Build history of the part. All positions in model axes, mm. A direction names the side the tool comes from. Coordinates: 2 decimals unless noted, no trailing zeros. Write each loop counter-clockwise with the first axis right and the second up, starting at its lowest first coordinate (ties: lowest second). Pieces come first, ordered by that corner, then holes.
```python
from build123d import *

# Parameters (mm, degrees)
BASE_PLATE_SKETCH_145X72_W  = 145
BASE_PLATE_SKETCH_145X72_H  = 72
BASE_PLATE_25_THICK_DEPTH   = 25
UNDERSIDE_RELIEF_SKETCH_W   = 72
UNDERSIDE_RELIEF_SKETCH_H   = 6
UNDERSIDE_RELIEF_CUT_DEPTH  = 50
CLEVIS_SLOT_CUT_DEPTH       = 50
LOCATING_PAD_SKETCH_W       = 12
LOCATING_PAD_SKETCH_H       = 72
LOCATING_PAD_5_HIGH_DEPTH   = 5
UPRIGHT_BLOCK_72_WIDE_DEPTH = 72
COUNTERBORE_SKETCH_36_R     = 28
COUNTERBORE_36X12_DEPTH     = 12
CROSS_HOLE_SKETCH_24_R      = 12
CROSS_HOLE_24_DEPTH         = 160.32670837


with BuildPart() as part:
    # Base Plate Sketch 145x72 → Base Plate 25 Thick (new body)
    with BuildSketch(Plane(origin=(0, 0, 0), x_dir=(1, 0, 0), z_dir=(0, 1, 0))):
        Rectangle(BASE_PLATE_SKETCH_145X72_W, BASE_PLATE_SKETCH_145X72_H)
    extrude(amount=BASE_PLATE_25_THICK_DEPTH)

    # Underside Relief Sketch → Underside Relief Cut (cut)
    with BuildSketch(Plane.XY.offset(36)):
        with Locations((-36.5, 3)):
            Rectangle(UNDERSIDE_RELIEF_SKETCH_W, UNDERSIDE_RELIEF_SKETCH_H)
    extrude(amount=-UNDERSIDE_RELIEF_CUT_DEPTH, mode=Mode.SUBTRACT)

    # Clevis Slot Sketch 24 Wide → Clevis Slot Cut (cut)
    with BuildSketch(Plane(origin=(0, 25, 0), x_dir=(1, 0, 0), z_dir=(0, 1, 0))):
        with BuildLine():
            Line((22.5, 12), (72.5, 12))
            Line((72.5, 12), (72.5, -12))
            Line((72.5, -12), (22.5, -12))
            ThreePointArc((22.5, -12), (10.5, 0), (22.5, 12))
        make_face()
    extrude(amount=-CLEVIS_SLOT_CUT_DEPTH, mode=Mode.SUBTRACT)

    # Locating Pad Sketch → Locating Pad 5 High (add)
    with BuildSketch(Plane(origin=(0, 25, 0), x_dir=(1, 0, 0), z_dir=(0, 1, 0))):
        with Locations((-66.5, 0)):
            Rectangle(LOCATING_PAD_SKETCH_W, LOCATING_PAD_SKETCH_H)
    extrude(amount=LOCATING_PAD_5_HIGH_DEPTH)

    # Upright Block Profile Sketch → Upright Block 72 Wide (add)
    with BuildSketch(Plane.XY.offset(36)):
        Polygon((-60.5, 25), (-60.5, 56), (-72.5, 56), (-72.5, 80), (-36.5, 80), (-36.5, 25), align=None)
    extrude(amount=-UPRIGHT_BLOCK_72_WIDE_DEPTH)

    # Counterbore Sketch Ø36 → Counterbore Ø36x12 (cut)
    with BuildSketch(Plane.ZY.offset(72.5)):
        with Locations((0, 42)):
            Circle(COUNTERBORE_SKETCH_36_R)
    extrude(amount=-COUNTERBORE_36X12_DEPTH, mode=Mode.SUBTRACT)

    # Cross Hole Sketch Ø24 → Cross Hole Ø24 (cut, through all)
    with BuildSketch(Plane.ZY.offset(60.5)):
        with Locations((0, 42)):
            Circle(CROSS_HOLE_SKETCH_24_R)
    extrude(amount=-CROSS_HOLE_24_DEPTH, mode=Mode.SUBTRACT)


solid = part.part
```
1. 3-axis set-ups, long thin cutter, end or side, ignore diameter. For faces 4 (the face through (47, 13, -12)), 5 (the face through (-67, 70, 0)), 6 (the face through (-37, 6, 11)): which of +Z, -Z, +X, -X, +Y, -Y reach the whole face in a straight line?
Computed values:
face 4: +X, +Y, -Y
face 5: -X
face 6: +Z, -X, -Y
2. Saw through at A-A on z = 0. List the corners of the cut face in (x, y), plus the area to 4 significant figures.
Computed values:
outline: (-72.5, 6) - (-0.5, 6) - (-0.5, 0) - (10.5, 0) - (10.5, 25) - (-36.5, 25) - (-36.5, 30) - (-60.5, 30) - (-60.5, 14) - (-72.5, 14) - close; (-72.5, 70) - (-60.5, 70) - (-60.5, 54) - (-36.5, 54) - (-36.5, 80) - (-72.5, 80) - close
area: 2,375 mm2
3. Probe line 1 along Y through (x, z) = (-45.5, 0); line 2 along Z through (x, y) = (23.5, 17.5); line 3 along X through (y, z) = (46, 15). List the from-to ranges inside material, lowest first.
Computed values:
line 1: y = 6 to 30, 54 to 80
line 2: z = -36 to -12, 12 to 36
line 3: x = -60.5 to -36.5
4. Saw through at B-B on y = 42. List the corners of the cut face in (x, z), plus the area to 3 significant figures.
Computed values:
outline: (-60.5, -36) - (-36.5, -36) - (-36.5, -12) - (-60.5, -12) - close; (-60.5, 12) - (-36.5, 12) - (-36.5, 36) - (-60.5, 36) - close
area: 1,150 mm2
5. Saw through at D-D on z = -28. List the corners of the cut face in (x, y), plus the area to 3 significant figures.
Computed values:
outline: (-72.5, 0) - (72.5, 0) - (72.5, 25) - (-36.5, 25) - (-36.5, 80) - (-72.5, 80) - (-72.5, 56) - (-60.5, 56) - (-60.5, 30) - (-72.5, 30) - close
area: 5,290 mm2
6. Flat gauge pins, fed straight in: pin 1 (1 mm diameter, centred on x = -29, z = 7.5, fed in from -Y); pin 2 (16.5 mm diameter, centred on y = 41, z = -2, fed in from +X); pin 3 (6 mm diameter, centred on y = 61, z = 0, fed in from +X); pin 4 (1.8 mm diameter, centred on y = 4, z = -1, fed in from -X). Where does each tip first touch, or does it go through?
Computed values:
pin 1: stops at y = 6
pin 2: passes through
pin 3: stops at x = -36.5
pin 4: stops at x = -0.5
7. Saw through at C-C on x = 42.5. List the corners of the cut face in (y, z).
Computed values:
outline: (0, -36) - (25, -36) - (25, -12) - (0, -12) - close; (0, 12) - (25, 12) - (25, 36) - (0, 36) - close
8. Mould opens along Y. For faces 1 (the face through (-67, 14, 0)), 2 (the face through (-37, 3, -14)), 3 (the face through (5, 25, -1)) say: +Y half, -Y half, draft (parallel to the pull), parting line (faces both ways), or undercut.
Computed values:
face 1: undercut
face 2: draft
face 3: +Y half
